For this review, take the finished solid that the model builds, in its own axes (mm). Face numbers are marked on the shaded views. A direction names the side the tool comes from. Round coordinates to 2 decimals unless told otherwise and drop trailing zeros. Order: outer loops, then holes, each group sorted by start corner. A loop starts at its lowest first (then second) coordinate and runs counter-clockwise, first axis right, second up. Notation, with made-up numbers: (9.25, 14.25) -> (62.25, 14.25) arc R20 ccw to (62.25, 30.25) -> close; hole circle Ø5 at (41, 19.5). An arc over 180 degrees is marked (long way). Use a Markdown table: item, result. Add a question column.
1) Consider section A-A (x = 0). State the section outline as (y, z) points, plus the area to 3 significant figures.
2) Consider section C-C (z = 26.5). State the section outline as (x, y) points, plus the area to 3 significant figures.
3) Clearance check with flat-ended pins moving along their axes: P1, Ø3, axis at x = -2.5, z = 11.5, coming from the +Y side; P2, Ø4, axis at x = 6, z = 27.5, coming from the +Y side; P3, Ø10, axis at y = -3, z = 17, coming from the -X side; P4, Ø6, axis at x = -7.5, z = 41, coming from the +Y side. State where each tip first meets the part, or that it passes through.
4) Machinability: for the marked faces 1 and 2, which of the approach directions +Z, -Z, +X, -X, +Y, -Y give a long, thin tool a straight path to every point of the face, cutting with its end or side? Answer none if there is none.
5) Wall thickness on line 1 along Z through (x, y) = (2.5, -7); line 2 along X through (y, z) = (1.25, 7.5); line 3 along X through (y, z) = (-8.5, 33): over which ranges is each line inside the solid? List them lowest first. Write a range as [from, to].
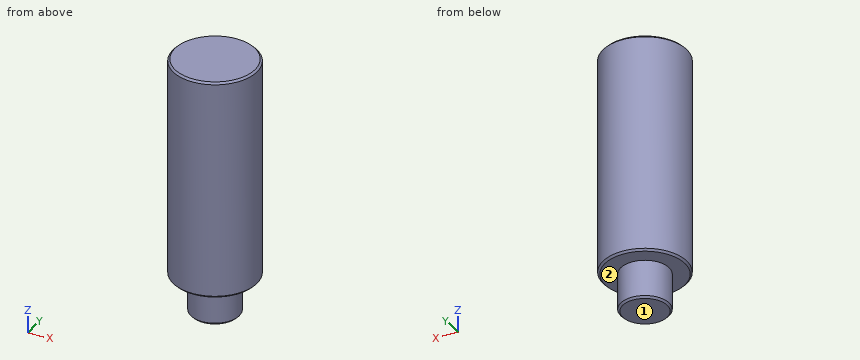
```python
from build123d import *

# Parameters (mm, degrees)
SKETCH1_R           = 6.35
BOSS_EXTRUDE1_DEPTH = 10
SKETCH2_R           = 11
BOSS_EXTRUDE2_DEPTH = 58
CHAMFER1_SIZE       = 0.5


with BuildPart() as part:
    # Sketch1 → Boss-Extrude1 (new body)
    with BuildSketch(Plane.XY):
        Circle(SKETCH1_R)
    extrude(amount=BOSS_EXTRUDE1_DEPTH)

    # Sketch2 → Boss-Extrude2 (add)
    with BuildSketch(Plane.XY.offset(10)):
        Circle(SKETCH2_R)
    extrude(amount=BOSS_EXTRUDE2_DEPTH)

    # Chamfer1
    chamfer1_edges = [part.edges().sort_by_distance(p)[0] for p in [
        (-6.35, 0, 0),
        (-11, 0, 10),
        (-11, 0, 68),
    ]]
    chamfer(chamfer1_edges, length=CHAMFER1_SIZE)


solid = part.part
```
Results list:
| question | item | result |
|---|---|---|
| 1 | outline | (-11, 10.5) -> (-10.5, 10) -> (-6.35, 10) -> (-6.35, 0.5) -> (-5.85, 0) -> (5.85, 0) -> (6.35, 0.5) -> (6.35, 10) -> (10.5, 10) -> (11, 10.5) -> (11, 67.5) -> (10.5, 68) -> (-10.5, 68) -> (-11, 67.5) -> close |
| 1 | area | 1,400 mm2 |
| 2 | outline | circle Ø22 at (0, 0) |
| 2 | area | 380 mm2 |
| 3 | P1 | y = 10.95 |
| 3 | P2 | y = 10.25 |
| 3 | P3 | x = -11 |
| 3 | P4 | y = 10.04 |
| 4 | face 1 | -Z, +X, -X, +Y, -Y |
| 4 | face 2 | -Z |
| 5 | line 1 | [10, 68] |
| 5 | line 2 | [-6.23, 6.23] |
| 5 | line 3 | [-6.98, 6.98] |
